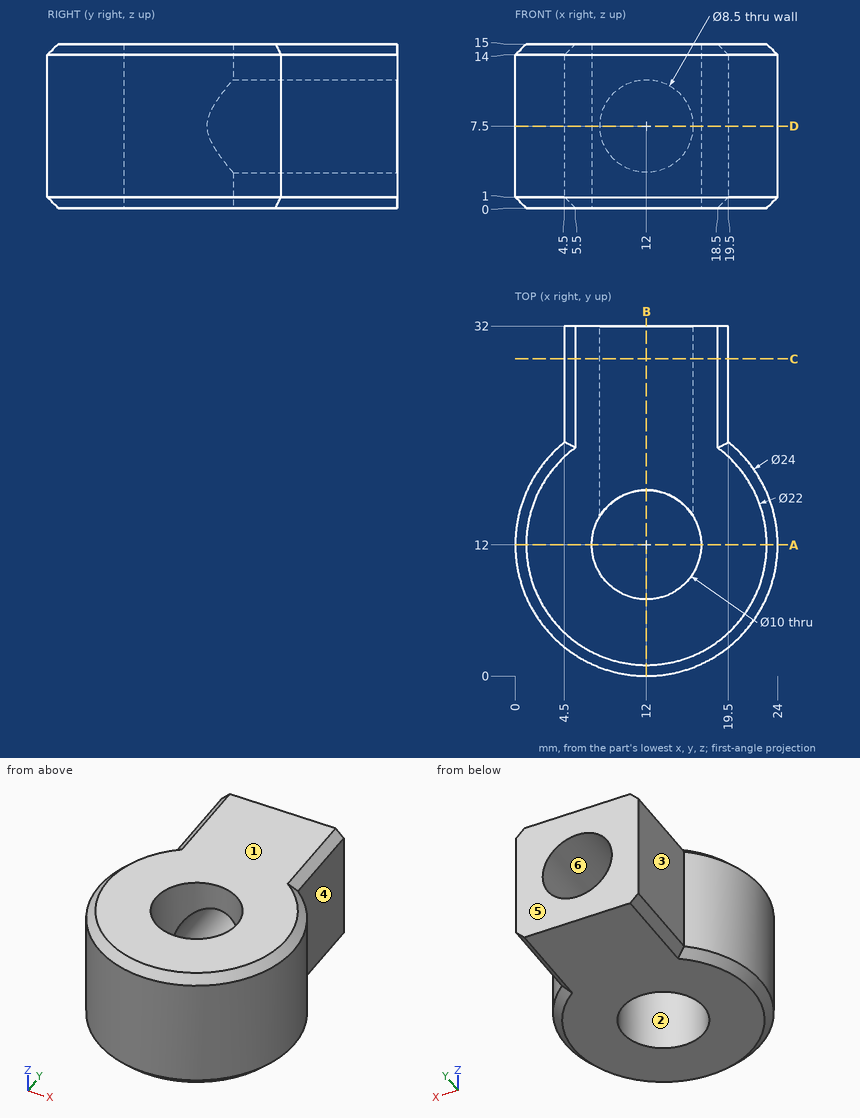
Source: three-view drawing plus pictorial views. Frame: mm from the lowest corner of the part. A direction names the side the tool comes from. Give positions to 0.01 mm unless a question says otherwise; leave off trailing zeros. Order: outer loops, then holes, each group sorted by start corner. A loop starts at its lowest first (then second) coordinate and runs counter-clockwise, first axis right, second up. Notation, with made-up numbers: (9.5, -17.75) -> (33.5, -17.75) arc R12 cw to (33.5, 2.25) -> close; hole circle Ø6 at (73, -4.75). An arc over 180 degrees is marked (long way). Use a Markdown table: item, result.
Q1. Access query for the marked faces 4, 5 and 6. Directions: +Z, -Z, +X, -X, +Y, -Y. A direction counts if a zero-diameter tool reaches every point of the face in a straight line with its end or side. Return the directions, or none.
A:
| item | result |
|---|---|
| face 4 | +Z, -Z, +X, +Y |
| face 5 | +Z, -Z, +X, -X, +Y |
| face 6 | +Y |
Q2. First-contact query: P1, Ø2, axis at y = 14.5, z = 7, coming from the +X side; P2, Ø2, axis at x = 10, y = 15, coming from the +Z side; P3, Ø1, axis at x = 20, z = 10, coming from the -Y side; P4, Ø3, axis at y = 24.5, z = 5.5, coming from the +X side. Flat tips, straight axial feed; report the tip coordinate or a pass-through.
A:
| item | result |
|---|---|
| P1 | x = 23.91 |
| P2 | through |
| P3 | y = 2.63 |
| P4 | x = 19.5 |
Q3. Section B-B (x = 12). Return the cut outline in (y, z), and give its area (4 significant figures).
A:
| item | result |
|---|---|
| outline | (0, 1) -> (1, 0) -> (7, 0) -> (7, 15) -> (1, 15) -> (0, 14) -> close; (17, 0) -> (32, 0) -> (32, 3.25) -> (17, 3.25) -> close; (17, 11.75) -> (32, 11.75) -> (32, 15) -> (17, 15) -> close |
| area | 201.5 mm^2 |
Q4. Pull-direction query (X, two-part tool) for the marked faces 1, 2 and 3; classes: +X half, -X half, draft (parallel to the pull), parting line (faces both ways), or undercut.
A:
| item | result |
|---|---|
| face 1 | draft |
| face 2 | undercut |
| face 3 | -X half |
Q5. Material intervals for line 1 (Z direction, x = 12, y = 28); line 2 (X direction, y = 20, z = 8.25); line 3 (Z direction, x = 13.75, y = 19), sorted ascending. Write a range as [from, to].
A:
| item | result |
|---|---|
| line 1 | [0, 3.25], [11.75, 15] |
| line 2 | [3.06, 7.82], [16.18, 20.94] |
| line 3 | [0, 3.63], [11.37, 15] |
Q6. Section C-C (y = 29). Return the cut outline in (x, z), and give its area (3 significant figures).
A:
| item | result |
|---|---|
| outline | (4.5, 1) -> (5.5, 0) -> (18.5, 0) -> (19.5, 1) -> (19.5, 14) -> (18.5, 15) -> (5.5, 15) -> (4.5, 14) -> close; hole circle Ø8.5 at (12, 7.5) |
| area | 166 mm^2 |
Q7. Section D-D (z = 7.5). Return the cut outline in (x, y), and give its area (3 significant figures).
A:
| item | result |
|---|---|
| outline | (4.5, 21.37) arc R12 ccw (long way) to (19.5, 21.37) -> (19.5, 32) -> (16.25, 32) -> (16.25, 14.63) arc R5 cw (long way) to (7.75, 14.63) -> (7.75, 32) -> (4.5, 32) -> close |
| area | 373 mm^2 |
Q8. Section A-A (y = 12). Return the cut outline in (x, z), and give its area (3 significant figures).
A:
| item | result |
|---|---|
| outline | (0, 1) -> (1, 0) -> (7, 0) -> (7, 15) -> (1, 15) -> (0, 14) -> close; (17, 0) -> (23, 0) -> (24, 1) -> (24, 14) -> (23, 15) -> (17, 15) -> close |
| area | 208 mm^2 |
